Geometry check sheet. Reference: the model listing, model coordinates, mm. Face numbers are marked on the shaded views. Round coordinates to 2 decimals unless told otherwise and drop trailing zeros. Loops run counter-clockwise (first coordinate to the right, second up) from the corner with the lowest first, then second, coordinate; pieces in that order, holes last. Notation, with made-up numbers: (-25.5, -33.75) - (18.5, -33.75) arc R20 ccw to (18.5, -5.75) - close; hole circle Ø5 at (63, 49.25). An arc over 180 degrees is marked (long way). Answer as CSV lines item,"result". Start each with the question number.
1) Cross-section at A-A on x = 0. Record the boundary of the cut face in (y, z), and give its area (3 significant figures).
2) Draft check along X on the marked faces 1, 2, 3 and 4. Enter one of: released by +X, released by -X, zero draft, split by the parting line, or undercut.
3) Cross-section at B-B on z = 0. Record the boundary of the cut face in (x, y).
4) Cross-section at D-D on x = 52.5. Record the boundary of the cut face in (y, z), and give its area (3 significant figures).
5) Cross-section at C-C on y = 2. Record the boundary of the cut face in (x, z), and give its area (3 significant figures).
6) Thickness scan on line 1 along X through (y, z) = (-10, -5); line 2 along X through (y, z) = (-9, 0); line 3 along Z through (x, y) = (-36, -1.5). Record the ranges inside material, lowest first.
from build123d import *

# Parameters (mm, degrees)
SKETCH_1_W               = 120
SKETCH_1_H               = 120
EXTRUDE_1_DEPTH          = 21
CUT_EXTRUDE_1_DEPTH      = 95.678403028
CUT_EXTRUDE_1_DEPTH_BACK = 95.678403028
SKETCH_2_R               = 55
SKETCH_2_R_2             = 2.25


with BuildPart() as part:
    # 草图1 → 凸台-拉伸1 (new, symmetric)
    with BuildSketch(Plane(origin=(0, 0, 0), x_dir=(1, 0, 0), z_dir=(0, 1, 0))):
        Rectangle(SKETCH_1_W, SKETCH_1_H)
    extrude(amount=EXTRUDE_1_DEPTH, both=True)

    # 草图2 → 切除-拉伸1 (cut, two sides: drawn at the far end of the back side and taken through both)
    with BuildSketch(Plane(origin=(0, 21, 0), x_dir=(1, 0, 0), z_dir=(0, 1, 0)).offset(-CUT_EXTRUDE_1_DEPTH_BACK)):
        with Locations(Location((0, 0, 0), (0, 0, 270))):
            Circle(SKETCH_2_R)
        with Locations(Location((-52.5, 52.5, 0), (0, 0, 270))):
            Circle(SKETCH_2_R_2)
        with Locations(Location((52.5, 52.5, 0), (0, 0, 270))):
            Circle(SKETCH_2_R_2)
        with Locations(Location((52.5, -52.5, 0), (0, 0, 270))):
            Circle(SKETCH_2_R_2)
        with Locations(Location((-52.5, -52.5, 0), (0, 0, 270))):
            Circle(SKETCH_2_R_2)
    extrude(amount=CUT_EXTRUDE_1_DEPTH + CUT_EXTRUDE_1_DEPTH_BACK, mode=Mode.SUBTRACT)


solid = part.part
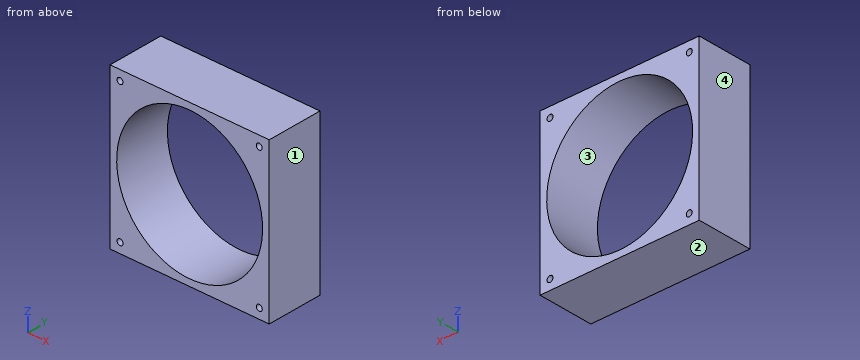
Answer block:
1,outline,"(-21, -60) - (21, -60) - (21, -55) - (-21, -55) - close; (-21, 55) - (21, 55) - (21, 60) - (-21, 60) - close"
1,area,"420 mm^2"
2,face 1,"released by +X"
2,face 2,"zero draft"
2,face 3,"undercut"
2,face 4,"released by -X"
3,outline,"(-60, -21) - (-55, -21) - (-55, 21) - (-60, 21) - close; (55, -21) - (60, -21) - (60, 21) - (55, 21) - close"
4,outline,"(-21, -60) - (21, -60) - (21, -54.75) - (-21, -54.75) - close; (-21, -50.25) - (21, -50.25) - (21, -16.39) - (-21, -16.39) - close; (-21, 16.39) - (21, 16.39) - (21, 50.25) - (-21, 50.25) - close; (-21, 54.75) - (21, 54.75) - (21, 60) - (-21, 60) - close"
4,area,"3,280 mm^2"
5,outline,"(-60, -60) - (60, -60) - (60, 60) - (-60, 60) - close; hole circle Ø110 at (0, 0); hole circle Ø4.5 at (-52.5, -52.5); hole circle Ø4.5 at (-52.5, 52.5); hole circle Ø4.5 at (52.5, -52.5); hole circle Ø4.5 at (52.5, 52.5)"
5,area,"4,830 mm^2"
6,line 1,"x = -60 to -54.77, 54.77 to 60"
6,line 2,"x = -60 to -55, 55 to 60"
6,line 3,"z = -60 to -41.58, 41.58 to 60"
